The model under review builds one solid part; all positions refer to its coordinate system, in mm. Face numbers are marked on the shaded views. A direction names the side the tool comes from. Round coordinates to 2 decimals unless told otherwise and drop trailing zeros. Write each loop counter-clockwise with the first axis right and the second up, starting at its lowest first coordinate (ties: lowest second). Pieces come first, ordered by that corner, then holes.
Item 1: Add section B-B (z = 0). Give the boundary of the cut face in (x, y).
Item 2: Clearance check with flat-ended pins moving along their axes: pin 1 Ø12 at (x, y) = (-11.5, 33) entering from -Z; pin 2 Ø10 at (y, z) = (36.5, -4.5) entering from +X; pin 3 Ø12 at (y, z) = (39, -3) entering from -X; pin 4 Ø11 at (x, z) = (-8.5, -3) entering from -Y. State where each tip first meets the part, or that it passes through.
Item 3: Machinability: for the marked faces 4, 5 and 6, which of the approach directions +Z, -Z, +X, -X, +Y, -Y give a long, thin tool a straight path to every point of the face, cutting with its end or side? Answer none if there is none.
Item 4: Draft analysis for pull direction X (two halves, no side actions). For the marked faces 1, 2 and 3, state which applies: +X half, -X half, draft (parallel to the pull), parting line (faces both ways), or undercut.
Item 5: Add section C-C (y = 9). Give the boundary of the cut face in (x, z), plus the area to 3 significant figures.
Item 6: Add section A-A (x = 0). Give the boundary of the cut face in (y, z), plus the area to 3 significant figures.
Item 7: To check wall thickness, follow L1, parallel to X at y = 36, z = 0; L2, parallel to X at y = 47.75, z = 0; L3, parallel to Y at x = 5, z = 16. State the ranges of each line that lie inside material, in increasing order.
```python
from build123d import *

# Parameters (mm, degrees)
COUNTERBORE_SKETCH_12_R = 6
COUNTERBORE_12X1_DEPTH  = 1
BORE_SKETCH_10_R        = 5
BORE_10X47_DEPTH        = 47


with BuildPart() as part:
    # Nozzle Profile Sketch → Nozzle Body Revolve (revolve)
    with BuildSketch(Plane.XY, mode=Mode.PRIVATE) as nozzle_body_revolve_sk:
        Polygon((0, 0), (0, 48), (-12, 48), (-12, 43), (-18, 43), (-18, 38), (-12, 38), (-12, 8), (-6, 0), align=None)
    revolve(nozzle_body_revolve_sk.sketch.rotate(Axis((0, 0, 0), (0, 1, 0)), 270), axis=Axis((0, 0, 0), (0, 1, 0)))

    # Counterbore Sketch Ø12 → Counterbore Ø12x1 (cut)
    with BuildSketch(Plane(origin=(0, 48, 0), x_dir=(1, 0, 0), z_dir=(0, 1, 0))):
        with Locations(Location((0, 0, 0), (0, 0, 270))):
            Circle(COUNTERBORE_SKETCH_12_R)
    extrude(amount=-COUNTERBORE_12X1_DEPTH, mode=Mode.SUBTRACT)

    # Bore Sketch Ø10 → Bore Ø10x47 (cut)
    with BuildSketch(Plane(origin=(0, 47, 0), x_dir=(1, 0, 0), z_dir=(0, 1, 0))):
        with Locations(Location((0, 0, 0), (0, 0, 270))):
            Circle(BORE_SKETCH_10_R)
    extrude(amount=-BORE_10X47_DEPTH, mode=Mode.SUBTRACT)


solid = part.part
```
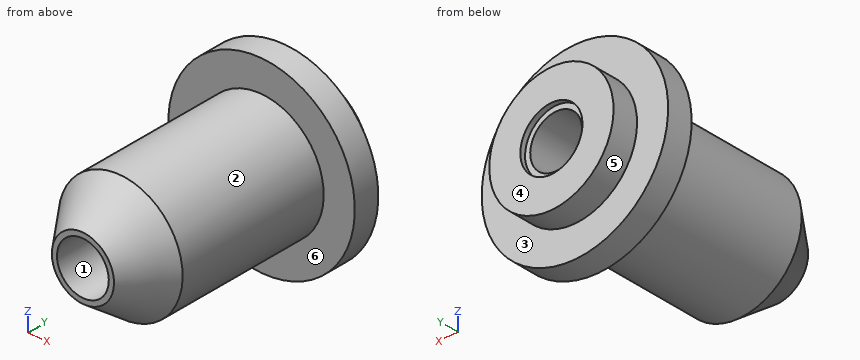
Numbers:
1. outline: (-18, 38) - (-12, 38) - (-12, 8) - (-6, 0) - (-5, 0) - (-5, 47) - (-6, 47) - (-6, 48) - (-12, 48) - (-12, 43) - (-18, 43) - close; (5, 0) - (6, 0) - (12, 8) - (12, 38) - (18, 38) - (18, 43) - (12, 43) - (12, 48) - (6, 48) - (6, 47) - (5, 47) - close
2. pin 1: stops at z = -16.03
2. pin 2: stops at x = 18
2. pin 3: stops at x = -18
2. pin 4: stops at y = 0
3. face 4: +Z, -Z, +X, -X, +Y
3. face 5: +Y
3. face 6: -Y
4. face 1: undercut
4. face 2: parting line
4. face 3: draft
5. outline: circle Ø24 at (0, 0); hole circle Ø10 at (0, 0)
5. area: 374 mm2
6. outline: (0, -6) - (8, -12) - (38, -12) - (38, -18) - (43, -18) - (43, -12) - (48, -12) - (48, -6) - (47, -6) - (47, -5) - (0, -5) - close; (0, 5) - (47, 5) - (47, 6) - (48, 6) - (48, 12) - (43, 12) - (43, 18) - (38, 18) - (38, 12) - (8, 12) - (0, 6) - close
6. area: 682 mm2
7. L1: x = -12 to -5, 5 to 12
7. L2: x = -12 to -6, 6 to 12
7. L3: y = 38 to 43
